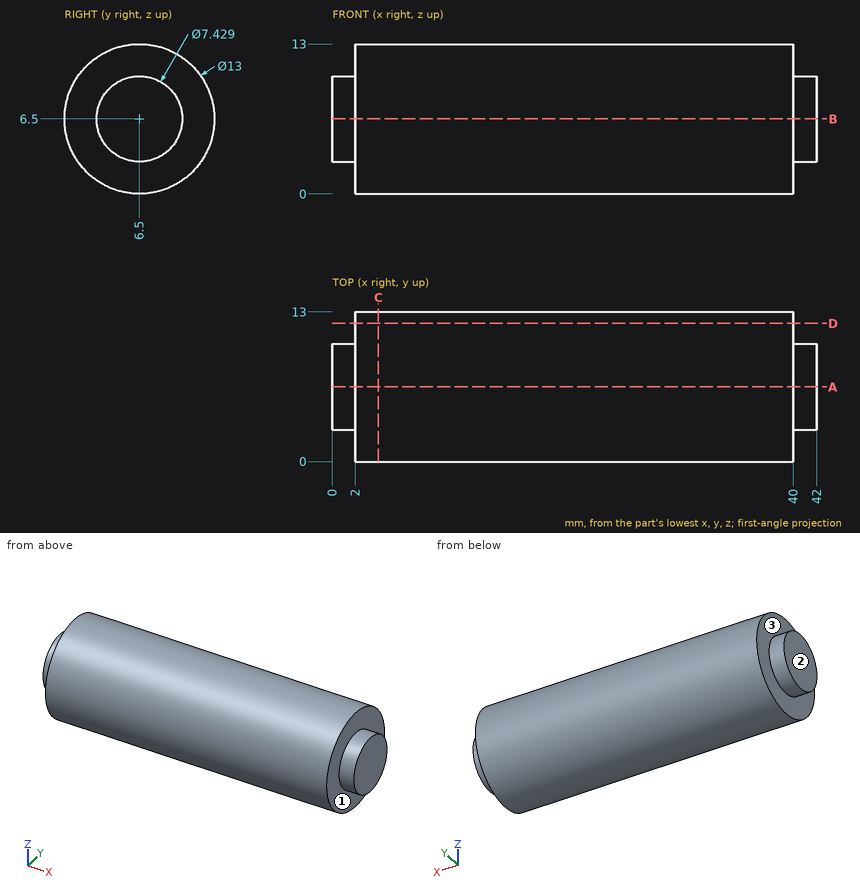
The figure shows three views and two pictorial views of one solid part (mm, origin at its lowest corner). Answer the questions. A direction names the side the tool comes from. Coordinates: 2 decimals unless noted, no trailing zeros. Loops run counter-clockwise (first coordinate to the right, second up) from the corner with the lowest first, then second, coordinate; pieces in that order, holes last.
1) Find section A-A on y = 6.5. Write down the section's boundary in (x, z) (1 decimal).
2) A tool of negligible diameter and unlimited length cuts with its end or side. For the marked faces 1, 2 and 3, from which of +Z, -Z, +X, -X, +Y, -Y can it reach the whole face along a straight path? Write none if from no direction.
3) Find section C-C on x = 4. Write down the section's boundary in (y, z), then the cut area to 3 significant figures.
4) Find the intervals of material crossed by L1, parallel to X at y = 8, z = 3; L2, parallel to Z at x = 28.5, y = 6.25 (1 decimal); L3, parallel to Z at x = 38.5, y = 4, in increasing order.
5) Find section D-D on y = 12. Write down the section's boundary in (x, z).
6) Flat-ended cylindrical pins translate along their axes: pin 1 Ø6 at (x, z) = (37.5, 11) entering from +Y (1 decimal); pin 2 Ø2 at (x, y) = (18, 3) entering from -Z; pin 3 Ø2 at (x, y) = (10, 5) entering from +Z. Find the tip coordinate at first contact, or state that the pin passes through.
Values:
1. outline: (0, 2.8) - (2, 2.8) - (2, 0) - (40, 0) - (40, 2.8) - (42, 2.8) - (42, 10.2) - (40, 10.2) - (40, 13) - (2, 13) - (2, 10.2) - (0, 10.2) - close
2. face 1: +X
2. face 2: +Z, -Z, -X, +Y, -Y
2. face 3: -X
3. outline: circle Ø13 at (6.5, 6.5)
3. area: 133 mm2
4. L1: x = 2 to 40
4. L2: z = 0 to 13
4. L3: z = 0.5 to 12.5
5. outline: (2, 3.04) - (40, 3.04) - (40, 9.96) - (2, 9.96) - close
6. pin 1: stops at y = 12.8
6. pin 2: stops at z = 0.5
6. pin 3: stops at z = 12.98
